from build123d import *

# Parameters (mm, degrees)
SKETCH1_R           = 4
BOSS_EXTRUDE1_DEPTH = 2
BOSS_EXTRUDE2_DEPTH = 1.5
SKETCH3_R           = 1.5
CUT_EXTRUDE1_DEPTH  = 8.375353099


with BuildPart() as part:
    # Sketch1 → Boss-Extrude1 (new body)
    with BuildSketch(Plane(origin=(0, 0, 0), x_dir=(1, 0, 0), z_dir=(0, 1, 0))):
        with Locations(Location((0, 0, 0), (0, 0, 270))):
            Circle(SKETCH1_R)
    extrude(amount=BOSS_EXTRUDE1_DEPTH)

    # Sketch2 → Boss-Extrude2 (add)
    with BuildSketch(Plane(origin=(0, 2, 0), x_dir=(1, 0, 0), z_dir=(0, 1, 0))):
        Polygon((0, 4.907477288), (-4.25, 2.453738644), (-4.25, -2.453738644), (0, -4.907477288), (4.25, -2.453738644), (4.25, 2.453738644), align=None)
    extrude(amount=BOSS_EXTRUDE2_DEPTH)

    # Sketch3 → Cut-Extrude1 (cut, through all)
    with BuildSketch(Plane(origin=(0, 3.5, 0), x_dir=(1, 0, 0), z_dir=(0, 1, 0))):
        with Locations(Location((0, 0, 0), (0, 0, 270))):
            Circle(SKETCH3_R)
    extrude(amount=-CUT_EXTRUDE1_DEPTH, mode=Mode.SUBTRACT)


solid = part.part
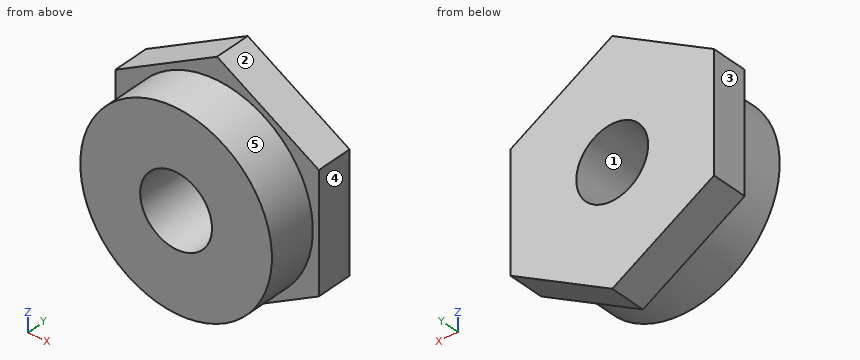
Check sheet for the modelled part. Datum: model origin and axes. Units: mm. Face numbers are marked on the shaded views. A direction names the side the tool comes from. Give positions to 0.01 mm unless a question says otherwise; leave off trailing zeros. Order: outer loops, then holes, each group sorted by start corner. A loop starts at its lowest first (then second) coordinate and runs counter-clockwise, first axis right, second up. Notation, with made-up numbers: M 7.25,-27 L 43.25,-27 A20 cw 43.25,5 Z; hole C -37.5,28.25 d1. An arc over 180 degrees is marked long. Answer as CSV lines item,"result". Start each with the question number.
Item 1: Tool access check on the marked faces 4 and 5. Record the directions out of +Z, -Z, +X, -X, +Y, -Y that give a thin tool (end or side, any length) a straight path to the whole face; none if there is none.
Item 2: Cross-section at A-A on z = 0. Enter the section's corners in (x, y), plus the area to 4 significant figures.
Item 3: Mould release check, pull along Z, two halves, no side actions. Record for the marked faces 1, 2 and 3: +Z half, -Z half, draft (parallel to the pull), parting line (faces both ways), or undercut.
Item 4: Cross-section at D-D on x = -2. Enter the section's corners in (y, z).
Item 5: Cross-section at C-C on x = -0.5. Enter the section's corners in (y, z), plus the area to 3 significant figures.
Item 6: Thickness scan on line 1 (X direction, y = 1.95, z = 0); line 2 (Z direction, x = 0.5, y = 1.05). Record the ranges inside material, lowest first. Write a range as [from, to].
Item 7: Cross-section at B-B on y = 2.15. Enter the section's corners in (x, z), plus the area to 3 significant figures.
Item 8: Gauge pin test, flat ends, axial feed: P1, Ø1.5, axis at x = -3.5, y = 0.5, coming from the +Z side; P2, Ø2, axis at x = -2.5, y = 1, coming from the +Z side. Record the tip position at first contact, or that the pin passes through.
Established:
1,face 4,"+Z, -Z, +X, +Y, -Y"
1,face 5,"-Y"
2,outline,"M -4.25,2 L -4,2 L -4,0 L -1.5,0 L -1.5,3.5 L -4.25,3.5 Z; M 1.5,0 L 4,0 L 4,2 L 4.25,2 L 4.25,3.5 L 1.5,3.5 Z"
2,area,"18.25 mm^2"
3,face 1,"undercut"
3,face 2,"+Z half"
3,face 3,"draft"
4,outline,"M 0,-3.46 L 2,-3.46 L 2,-3.75 L 3.5,-3.75 L 3.5,3.75 L 2,3.75 L 2,3.46 L 0,3.46 Z"
5,outline,"M 0,-3.97 L 2,-3.97 L 2,-4.62 L 3.5,-4.62 L 3.5,-1.41 L 0,-1.41 Z; M 0,1.41 L 3.5,1.41 L 3.5,4.62 L 2,4.62 L 2,3.97 L 0,3.97 Z"
5,area,"19.8 mm^2"
6,line 1,"x = [-4, -1.5], [1.5, 4]"
6,line 2,"z = [-3.97, -1.41], [1.41, 3.97]"
7,outline,"M -4.25,-2.45 L 0,-4.91 L 4.25,-2.45 L 4.25,2.45 L 0,4.91 L -4.25,2.45 Z; hole C 0,0 d3"
7,area,"55.5 mm^2"
8,P1,"stops at z = 2.9"
8,P2,"stops at z = 3.71"
